Geometry check sheet. Reference: the model listing, model coordinates, mm. A direction names the side the tool comes from. Coordinates: 2 decimals unless noted, no trailing zeros. Write each loop counter-clockwise with the first axis right and the second up, starting at its lowest first coordinate (ties: lowest second). Pieces come first, ordered by that corner, then holes.
from build123d import *

# Parameters (mm, degrees)
SKETCH1_W           = 50
SKETCH1_H           = 50
SKETCH1_W_2         = 46
SKETCH1_H_2         = 46
BOSS_EXTRUDE1_DEPTH = 600


with BuildPart() as part:
    # Sketch1 → Boss-Extrude1 (new body)
    with BuildSketch(Plane.XY):
        Rectangle(SKETCH1_W, SKETCH1_H)
        Rectangle(SKETCH1_W_2, SKETCH1_H_2, mode=Mode.SUBTRACT)
    extrude(amount=BOSS_EXTRUDE1_DEPTH)


solid = part.part
1. Sectioned sample at C-C, the plane z = 541.5. Record the boundary of the cut face in (x, y), and give its area (3 significant figures).
Computed values:
outline: (-25, -25) - (25, -25) - (25, 25) - (-25, 25) - close; hole (-23, -23) - (23, -23) - (23, 23) - (-23, 23) - close
area: 384 mm2
2. Gauge pin test, flat end, axial feed: pin 1 Ø8 at (x, y) = (-19.5, -18.5) entering from +Z. Record the tip position at first contact, or that the pin passes through.
Computed values:
pin 1: stops at z = 600
3. Thickness scan on line 1 along X through (y, z) = (-5.5, 470). Record the ranges inside material, lowest first.
Computed values:
line 1: x = -25 to -23, 23 to 25
4. Draft check along Y on faces 3 (the flat face through (-23, 0, 296)), 4 (the flat face through (0, 25, 296)), 5 (the flat face through (25, 0, 296)). Enter one of: released by +Y, released by -Y, zero draft, split by the parting line, or undercut.
Computed values:
face 3: undercut
face 4: released by +Y
face 5: zero draft
5. Sectioned sample at A-A, the plane y = -8. Record the boundary of the cut face in (x, z).
Computed values:
outline: (-25, 0) - (-23, 0) - (-23, 600) - (-25, 600) - close; (23, 0) - (25, 0) - (25, 600) - (23, 600) - close
6. Access from +Z, -Z, +X, -X, +Y, -Y to the whole of each face (thin tool, end or side, straight path). Record for faces 1 (the flat face through (0, -23, 296)), 2 (the flat face through (0, -25, 296)).
Computed values:
face 1: +Z, -Z
face 2: +Z, -Z, +X, -X, -Y
